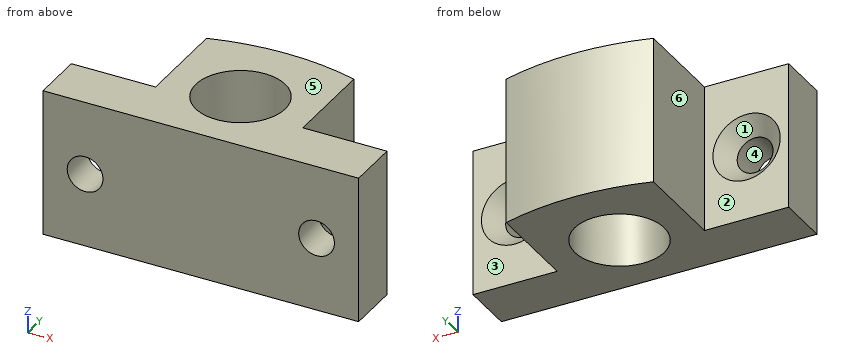
from build123d import *

# Parameters (mm, degrees)
EXTRUDE_1_DEPTH           = 7
HOLE_WIZARD_1_D           = 3.4
HOLE_WIZARD_1_CSINK_D     = 6.4
HOLE_WIZARD_1_CSINK_ANGLE = 90
SKETCH_5_R                = 4.25
CUT_EXTRUDE_1_DEPTH       = 26.416530054


with BuildPart() as part:
    # 草图1 → 凸台-拉伸1 (new, symmetric)
    with BuildSketch(Plane.XY):
        with BuildLine():
            Line((-15, 5), (-7, 5))
            Line((-7, 5), (-7, 14))
            ThreePointArc((-7, 14), (0, 15), (7, 14))
            Line((7, 14), (7, 5))
            Line((7, 5), (15, 5))
            Line((15, 5), (15, 0))
            Line((15, 0), (-15, 0))
            Line((-15, 0), (-15, 5))
        make_face()
    extrude(amount=EXTRUDE_1_DEPTH, both=True)

    # 打孔尺寸开槽半沉头螺钉的类型1 (through all)
    with Locations(Plane(origin=(0, 5, 0), x_dir=(1, 0, 0), z_dir=(0, 1, 0))):
        with Locations((-11, 0), (11, 0)):
            CounterSinkHole(HOLE_WIZARD_1_D / 2, HOLE_WIZARD_1_CSINK_D / 2, counter_sink_angle=HOLE_WIZARD_1_CSINK_ANGLE)

    # 草图5 → 切除-拉伸1 (cut, through all)
    with BuildSketch(Plane.XY.offset(7)):
        with Locations((0, 7)):
            Circle(SKETCH_5_R)
    extrude(amount=-CUT_EXTRUDE_1_DEPTH, mode=Mode.SUBTRACT)


solid = part.part
Geometry: final body of the model. Coordinates: model frame, mm. Face numbers are marked on the shaded views. A direction names the side the tool comes from. Coordinates: 2 decimals unless noted, no trailing zeros. Loops run counter-clockwise (first coordinate to the right, second up) from the corner with the lowest first, then second, coordinate; pieces in that order, holes last. Notation, with made-up numbers: (2, 9) - (17, 9) arc R5 ccw to (17, 15) - close; hole circle Ø2 at (58.5, 89). An arc over 180 degrees is marked (long way). One line per question, with ' | ' between items. Start each with the question number.
(1) Ray query, L1, parallel to Z at x = -11, y = 2.5; L2, parallel to X at y = 3.25, z = 0.75; L3, parallel to Y at x = -0.25, z = 4.25. Return the intervals inside material, ascending. Write a range as from..to.
(2) Cut plane C-C on x = 0. Output: boundary loops of the cut face in (y, z), and give its area (3 significant figures).
(3) First-contact query: pin 1 (2 mm diameter, centred on x = 3.5, z = -0.5, fed in from +Y); pin 2 (1.5 mm diameter, centred on y = 9.5, z = -1.5, fed in from -X); pin 3 (2.5 mm diameter, centred on y = 10.5, z = -0.5, fed in from +X). Flat tips, straight axial feed; report the tip coordinate or a pass-through.
(4) Cut plane A-A on z = 0. Output: boundary loops of the cut face in (x, y).
(5) Draft query along Z for the marked faces 4, 5 and 6. Return one class per face: +Z half, -Z half, draft (parallel to the pull), parting line (faces both ways), or undercut.
(6) Reachability of the marked faces 1, 2 and 3 from +Z, -Z, +X, -X, +Y, -Y: full face, straight path, thin tool, end or side. Return the list, or none.
(7) Cut plane D-D on z = 5.25. Output: boundary loops of the cut face in (x, y), and give its area (3 significant figures).
(8) Cut plane B-B on y = 7. Output: boundary loops of the cut face in (x, z).
Here are the results:
1) L1: -7..-1.7, 1.7..7 | L2: -15..-12.53, -9.47..-2, 2..9.47, 12.53..15 | L3: 0..2.76, 11.24..15
2) outline: (0, -7) - (2.75, -7) - (2.75, 7) - (0, 7) - close; (11.25, -7) - (15, -7) - (15, 7) - (11.25, 7) - close | area: 91.0 mm²
3) pin 1: y = 14.87 | pin 2: x = -7 | pin 3: x = 7
4) outline: (-15, 0) - (-12.7, 0) - (-12.7, 3.5) - (-14.2, 5) - (-15, 5) - close; (-9.3, 0) - (9.3, 0) - (9.3, 3.5) - (7.8, 5) - (7, 5) - (7, 14) arc R25 ccw to (-7, 14) - (-7, 5) - (-7.8, 5) - (-9.3, 3.5) - close; (12.7, 0) - (15, 0) - (15, 5) - (14.2, 5) - (12.7, 3.5) - close; hole circle Ø8.5 at (0, 7)
5) face 4: undercut | face 5: +Z half | face 6: draft
6) face 1: +Y | face 2: +Z, -Z, -X, +Y | face 3: +Z, -Z, +X, +Y
7) outline: (-15, 0) - (15, 0) - (15, 5) - (7, 5) - (7, 14) arc R25 ccw to (-7, 14) - (-7, 5) - (-15, 5) - close; hole circle Ø8.5 at (0, 7) | area: 229 mm²
8) outline: (-7, -7) - (-4.25, -7) - (-4.25, 7) - (-7, 7) - close; (4.25, -7) - (7, -7) - (7, 7) - (4.25, 7) - close
